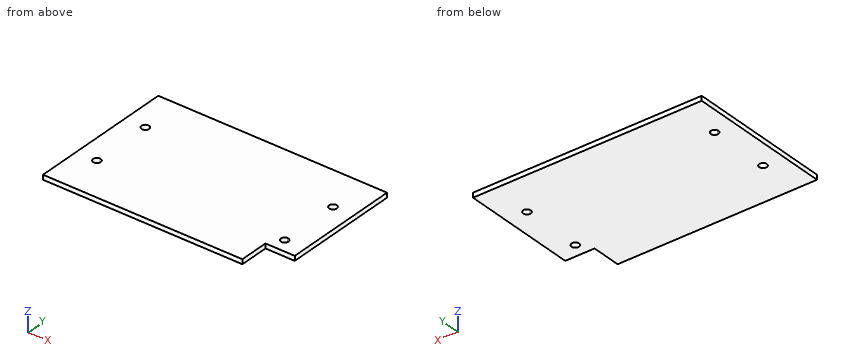
from build123d import *

# Parameters (mm, degrees)
SKETCH_1_W          = 390
SKETCH_1_H          = 250
EXTRUDE_1_DEPTH     = 8
CUT_EXTRUDE_1_DEPTH = 8
SKETCH_3_W          = 50
SKETCH_3_H          = 50
CUT_EXTRUDE_2_DEPTH = 60


with BuildPart() as part:
    # Sketch 1 → Extrude 1 (new body)
    with BuildSketch(Plane.XY):
        with Locations((195, 125)):
            Rectangle(SKETCH_1_W, SKETCH_1_H)
    extrude(amount=EXTRUDE_1_DEPTH)

    # Sketch 2 → Cut-Extrude 1 (cut)
    with BuildSketch(Plane.XY.offset(8)):
        with BuildLine():
            ThreePointArc((41.5, 177.5), (30.403805922, 182.096194078), (35, 171))
            Line((35, 171), (35, 177.5))
            Line((35, 177.5), (41.5, 177.5))
        make_face()
        with BuildLine():
            Line((35, 177.5), (35, 171))
            ThreePointArc((35, 171), (39.596194078, 172.903805922), (41.5, 177.5))
            Line((41.5, 177.5), (35, 177.5))
        make_face()
        with BuildLine():
            Line((35, 79), (35, 72.5))
            Line((35, 72.5), (41.5, 72.5))
            ThreePointArc((41.5, 72.5), (39.596194078, 77.096194078), (35, 79))
        make_face()
        with BuildLine():
            Line((41.5, 72.5), (35, 72.5))
            Line((35, 72.5), (35, 79))
            ThreePointArc((35, 79), (30.403805922, 67.903805922), (41.5, 72.5))
        make_face()
        with BuildLine():
            ThreePointArc((355, 79), (350.403805922, 77.096194078), (348.5, 72.5))
            Line((348.5, 72.5), (355, 72.5))
            Line((355, 72.5), (355, 79))
        make_face()
        with BuildLine():
            Line((355, 72.5), (348.5, 72.5))
            ThreePointArc((348.5, 72.5), (355, 66), (361.5, 72.5))
            ThreePointArc((361.5, 72.5), (359.596194078, 77.096194078), (355, 79))
            Line((355, 79), (355, 72.5))
        make_face()
        with BuildLine():
            ThreePointArc((348.5, 177.5), (350.403805922, 172.903805922), (355, 171))
            Line((355, 171), (355, 177.5))
            Line((355, 177.5), (348.5, 177.5))
        make_face()
        with BuildLine():
            Line((355, 177.5), (355, 171))
            ThreePointArc((355, 171), (359.596194078, 172.903805922), (361.5, 177.5))
            ThreePointArc((361.5, 177.5), (355, 184), (348.5, 177.5))
            Line((348.5, 177.5), (355, 177.5))
        make_face()
    extrude(amount=-CUT_EXTRUDE_1_DEPTH, mode=Mode.SUBTRACT)

    # Sketch 3 → Cut-Extrude 2 (cut)
    with BuildSketch(Plane.XY.offset(8)):
        with Locations((365, 25)):
            Rectangle(SKETCH_3_W, SKETCH_3_H)
    extrude(amount=-CUT_EXTRUDE_2_DEPTH, mode=Mode.SUBTRACT)


solid = part.part
The model under review builds one solid part; all positions refer to its coordinate system, in mm. Give positions to 0.01 mm unless a question says otherwise; leave off trailing zeros. Loops run counter-clockwise (first coordinate to the right, second up) from the corner with the lowest first, then second, coordinate; pieces in that order, holes last. Notation, with made-up numbers: (73.25, -14.5) -> (94.25, -14.5) arc R27 ccw to (94.25, 12.5) -> close; hole circle Ø3 at (36.5, 75.25). An arc over 180 degrees is marked (long way). Answer as a JSON object with one key per item and string values. Group by question number.
Q1. Insertion check: pin 1 (2.5 mm diameter, centred on x = 363.5, z = 2.5, fed in from -Y). The pin has a flat end and moves straight along its axis. Give the tip position at first contact, or say it passes through.
Q2. Take a section at A-A (z = 1.5). Write out the cut boundary in (x, y), plus the area to 3 significant figures.
Q3. Wall thickness on line 1 along Y through (x, z) = (35, 6.25); line 2 along X through (y, z) = (72.5, 3.5); line 3 along X through (y, z) = (22.5, 2): over which ranges is each line inside the solid? List them lowest first.
Answer below:
{
 "1": {"pin 1": "stops at y = 50"},
 "2": {"outline": "(0, 0) -> (340, 0) -> (340, 50) -> (390, 50) -> (390, 250) -> (0, 250) -> close; hole circle Ø13 at (35, 72.5); hole circle Ø13 at (35, 177.5); hole circle Ø13 at (355, 72.5); hole circle Ø13 at (355, 177.5)", "area": "94,500 mm2"},
 "3": {"line 1": "y = 0 to 66, 79 to 171, 184 to 250", "line 2": "x = 0 to 28.5, 41.5 to 348.5, 361.5 to 390", "line 3": "x = 0 to 340"}
}
